```python
from build123d import *

# Parameters (mm, degrees)
PIN_BOSS_RELIEF_SKETCH_R = 18
PIN_BOSS_RELIEF_36_DEPTH = 17
WRIST_PIN_BORE_SKETCH_R  = 11
WRIST_PIN_BORE_DEPTH     = 157


with BuildPart() as part:
    # Piston Profile Sketch → Piston Body (revolve)
    with BuildSketch(Plane(origin=(0, 0, 0), x_dir=(1, 0, 0), z_dir=(0, 1, 0))):
        with BuildLine():
            ThreePointArc((0, 68), (23.091806354, 67.907697429), (46, 65))
            Line((46, 65), (42, 65))
            Line((42, 65), (42, 63))
            Line((42, 63), (46, 63))
            Line((46, 63), (46, 60))
            Line((46, 60), (42, 60))
            Line((42, 60), (42, 57))
            Line((42, 57), (46, 57))
            Line((46, 57), (46, 55))
            Line((46, 55), (42, 55))
            Line((42, 55), (42, 52))
            Line((42, 52), (46, 52))
            Line((46, 52), (46, 50))
            Line((46, 50), (42, 50))
            Line((42, 50), (42, 47))
            Line((42, 47), (46, 47))
            Line((46, 47), (46, 45))
            Line((46, 45), (42, 45))
            Line((42, 45), (42, 10.377701479))
            Line((42, 10.377701479), (42, 10))
            Line((42, 10), (46, 10))
            Line((46, 10), (46, 7))
            Line((46, 7), (42, 7))
            Line((42, 7), (42, 5))
            Line((42, 5), (46, 5))
            Line((46, 5), (46, 0))
            Line((46, 0), (0, 0))
            Line((0, 0), (0, 68))
        make_face()
    revolve(axis=Axis((0, 0, 0), (0, 0, -1)))

    # Pin Boss Relief Sketch → Pin Boss Relief Ø36 (cut)
    with BuildSketch(Plane(origin=(0, 42, 0), x_dir=(1, 0, 0), z_dir=(0, 1, 0))):
        with Locations(Location((0, 27, 0), (0, 0, 270))):
            Circle(PIN_BOSS_RELIEF_SKETCH_R)
    pin_boss_relief_36 = extrude(amount=-PIN_BOSS_RELIEF_36_DEPTH, mode=Mode.SUBTRACT)

    # Pin Boss Relief Mirror: Pin Boss Relief Ø36 across plane
    add(pin_boss_relief_36.mirror(Plane.ZX), mode=Mode.SUBTRACT)

    # Wrist Pin Bore Sketch → Wrist Pin Bore (cut)
    with BuildSketch(Plane(origin=(0, 25, 0), x_dir=(1, 0, 0), z_dir=(0, 1, 0))):
        with Locations(Location((0, 27, 0), (0, 0, 270))):
            Circle(WRIST_PIN_BORE_SKETCH_R)
    extrude(amount=-WRIST_PIN_BORE_DEPTH, mode=Mode.SUBTRACT)


solid = part.part
```
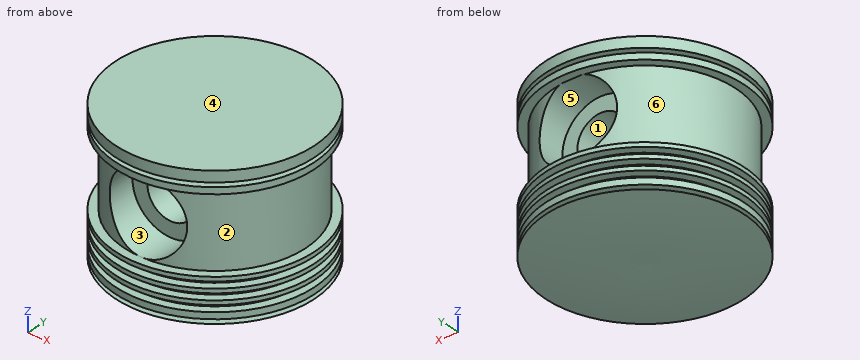
Design review of the part built by this model. Coordinates are the model's own, in mm. Face numbers are marked on the shaded views. A direction names the side the tool comes from. Give positions to 0.01 mm unless a question says otherwise; leave off trailing zeros. Order: outer loops, then holes, each group sorted by start corner. A loop starts at its lowest first (then second) coordinate and runs counter-clockwise, first axis right, second up. Notation, with made-up numbers: (11.25, -22) -> (59.25, -22) arc R19 cw to (59.25, -5) -> close; hole circle Ø8 at (60, 40.25). An arc over 180 degrees is marked (long way). Write item = value, one per line. Start each with the question number.
(1) We need section A-A on z = -21.5. Write out the cut boundary in (x, y), plus the area to 3 significant figures.
(2) We need section B-B on z = -41.5. Write out the cut boundary in (x, y), plus the area to 3 significant figures.
(3) To check wall thickness, follow line 1 along X through (y, z) = (-0.5, -27); line 2 along X through (y, z) = (-12, -27); line 3 along Y through (x, z) = (4, -9.5). State the ranges of each line that lie inside material, in increasing order.
(4) For the marked faces 1, 2 and 3, list the 3-axis set-ups (+Z, -Z, +X, -X, +Y, -Y) from which the entire face can be reached by the end or side of a thin tool; tool diameter is ignored.
(5) For pin 1 (1.1 mm diameter, centred on x = 3, z = -9.5, fed in from -Y); pin 2 (6 mm diameter, centred on y = -4.5, z = -33, fed in from -X); pin 3 (3 mm diameter, centred on y = 36.5, z = -27.5, fed in from -X); pin 4 (12 mm diameter, centred on x = 32, y = 25, fed in from +Z), all flat-tipped, find the tip position at first contact; note any pin that passes through.
(6) Mouldability with a two-part tool opening along Y and no side actions: class the marked faces 4, 5 and 6 as +Y half, -Y half, draft (parallel to the pull), parting line (faces both ways), or undercut.
Numbers:
q1.outline = (-17.14, -38.34) -> (-17.14, -25) -> (-9.53, -25) -> (-9.53, 25) -> (-17.14, 25) -> (-17.14, 38.34) arc R42 ccw to start; (9.53, -25) -> (17.14, -25) -> (17.14, -38.34) arc R42 ccw to (17.14, 38.34) -> (17.14, 25) -> (9.53, 25) -> close
q1.area = 3,510 mm^2
q2.outline = (-10.67, -40.62) -> (-10.67, -25) -> (10.67, -25) -> (10.67, -40.62) arc R42 ccw to (10.67, 40.62) -> (10.67, 25) -> (-10.67, 25) -> (-10.67, 40.62) arc R42 ccw to start
q2.area = 4,840 mm^2
q3.line_1 = -42 to -11, 11 to 42
q3.line_2 = -40.25 to -11, 11 to 40.25
q3.line_3 = -45.83 to -42, -25 to 25, 42 to 45.83
q4.face_1 = +Y, -Y
q4.face_2 = +X
q4.face_3 = none
q5.pin_1 = -45.93
q5.pin_2 = -41.97
q5.pin_3 = -23.22
q5.pin_4 = 0
q6.face_4 = draft
q6.face_5 = undercut
q6.face_6 = parting line
